```python
from build123d import *

# Parameters (mm, degrees)
CLAMP_RING_SKETCH_R          = 12.5
CLAMP_RING_25_DEPTH          = 13
CLAMP_BLOCK_DEPTH            = 13
BORE_SKETCH_R                = 6
BORE_12_DEPTH                = 13
COUNTERBORE_SKETCH_R         = 8
COUNTERBORE_16X2_DEPTH       = 2
MOUNTING_FLANGE_SKETCH_R     = 2.75
MOUNTING_FLANGE_2X_5_5_DEPTH = 7
CLAMP_SPLIT_SLOT_DEPTH       = 36.622441552
CLAMP_SCREW_HOLE_SKETCH_R    = 2.25
CLAMP_SCREW_HOLE_4_5_DEPTH   = 20


with BuildPart() as part:
    # Clamp Ring Sketch → Clamp Ring Ø25 (new body)
    with BuildSketch(Plane.XY):
        with Locations(Location((0, 0, 0), (0, 0, 180))):
            Circle(CLAMP_RING_SKETCH_R)
    extrude(amount=CLAMP_RING_25_DEPTH)

    # Clamp Block Sketch → Clamp Block (add)
    with BuildSketch(Plane.XY):
        with BuildLine():
            Line((-8.925, 22.5), (8.925, 22.5))
            Line((8.925, 22.5), (8.925, 8.751821239))
            ThreePointArc((8.925, 8.751821239), (0, 12.5), (-8.925, 8.751821239))
            Line((-8.925, 8.751821239), (-8.925, 22.5))
        make_face()
    extrude(amount=CLAMP_BLOCK_DEPTH)

    # Bore Sketch → Bore Ø12 (cut)
    with BuildSketch(Plane.XY.offset(13)):
        Circle(BORE_SKETCH_R)
    extrude(amount=-BORE_12_DEPTH, mode=Mode.SUBTRACT)

    # Counterbore Sketch → Counterbore Ø16x2 (cut)
    with BuildSketch(Plane.XY.offset(13)):
        Circle(COUNTERBORE_SKETCH_R)
    extrude(amount=-COUNTERBORE_16X2_DEPTH, mode=Mode.SUBTRACT)

    # Mounting Flange Sketch → Mounting Flange 2xØ5.5 (add)
    # profile 1 of 2: a face of its own
    with BuildSketch(Plane.XY):
        with BuildLine():
            Line((-8.925, 12.285952074), (-24.366131046, 3.44))
            Line((-24.366131046, 3.44), (-24.366131046, -3.437120562))
            Line((-24.366131046, -3.437120562), (-4.783542905, -11.548494156))
            ThreePointArc((-4.783542905, -11.548494156), (-12.247723806, -2.498651951), (-8.925, 8.751821239))
            Line((-8.925, 8.751821239), (-8.925, 12.285952074))
        make_face()
        with Locations((-18, 0)):
            Circle(MOUNTING_FLANGE_SKETCH_R, mode=Mode.SUBTRACT)
    # profile 2 of 2: a face of its own
    with BuildSketch(Plane.XY):
        with BuildLine():
            ThreePointArc((8.925, 8.751821239), (12.247723806, -2.498651951), (4.783542905, -11.548494156))
            Line((4.783542905, -11.548494156), (24.359179467, -3.44))
            Line((24.359179467, -3.44), (24.359179467, 3.44))
            Line((24.359179467, 3.44), (8.925, 12.285952074))
            Line((8.925, 12.285952074), (8.925, 8.751821239))
        make_face()
        with Locations((18, 0)):
            Circle(MOUNTING_FLANGE_SKETCH_R, mode=Mode.SUBTRACT)
    extrude(amount=MOUNTING_FLANGE_2X_5_5_DEPTH)

    # Split Slot Sketch → Clamp Split Slot (cut, through all)
    with BuildSketch(Plane.XY.offset(13)):
        with BuildLine():
            Line((0.5, 5.979130372), (0.5, 22.5))
            Line((0.5, 22.5), (-0.5, 22.5))
            Line((-0.5, 22.5), (-0.5, 5.979130372))
            ThreePointArc((-0.5, 5.979130372), (0, 6), (0.5, 5.979130372))
        make_face()
    extrude(amount=-CLAMP_SPLIT_SLOT_DEPTH, mode=Mode.SUBTRACT)

    # Clamp Screw Hole Sketch → Clamp Screw Hole Ø4.5 (cut)
    with BuildSketch(Plane(origin=(8.925, 0, 0), x_dir=(0, 0, -1), z_dir=(1, 0, 0))):
        with Locations((-6.5, 15.62591062)):
            Circle(CLAMP_SCREW_HOLE_SKETCH_R)
    extrude(amount=-CLAMP_SCREW_HOLE_4_5_DEPTH, mode=Mode.SUBTRACT)


solid = part.part
```
Can you work these out from the model? Positions are in its coordinate system, mm. A direction names the side the tool comes from. Round coordinates to 2 decimals unless told otherwise and drop trailing zeros. Loops run counter-clockwise (first coordinate to the right, second up) from the corner with the lowest first, then second, coordinate; pieces in that order, holes last. Notation, with made-up numbers: (-2, 26.25) -> (40, 26.25) arc R16 ccw to (40, 50.25) -> close; hole circle Ø9 at (18, -34.5). An arc over 180 degrees is marked (long way). Answer in a Markdown table with one row per item.
Item 1: Suppose I cut it at D-D, the plane x = 3.5. List the corners of the cut face in (y, z) for me, plus the area to 3 significant figures.
Answer block:
| item | result |
|---|---|
| outline | (-12, 0) -> (-4.87, 0) -> (-4.87, 11) -> (-7.19, 11) -> (-7.19, 13) -> (-12, 13) -> close; (4.87, 0) -> (22.5, 0) -> (22.5, 13) -> (7.19, 13) -> (7.19, 11) -> (4.87, 11) -> close; hole circle Ø4.5 at (15.63, 6.5) |
| area | 297 mm² |
Item 2: On a 3-axis mill with a long thin cutter (end or side, diameter ignored), from which of +Z, -Z, +X, -X, +Y, -Y can I reach the whole of each face in a straight line? I mean faces 5 (the flat face through (-2, -6, 11)), 6 (the flat face through (-14.712, -7.436, 3.451)). Say none if no direction works.
Answer block:
| item | result |
|---|---|
| face 5 | +Z |
| face 6 | +Z, -Z, -X, -Y |
Item 3: Suppose I cut it at B-B, the plane x = 18. List the corners of the cut face in (y, z) for me, plus the area to 3 significant figures.
Answer block:
| item | result |
|---|---|
| outline | (-6.07, 0) -> (-2.75, 0) -> (-2.75, 7) -> (-6.07, 7) -> close; (2.75, 0) -> (7.08, 0) -> (7.08, 7) -> (2.75, 7) -> close |
| area | 53.6 mm² |
Item 4: Will these pins go through, and if not, where does the flat tip stop? P1, Ø3, axis at y = 5.5, z = 10, coming from the -X side; P2, Ø3, axis at x = -6, z = 4, coming from the -Y side; P3, Ø19, axis at x = 0, y = 0, coming from the -Z side; P4, Ø1.5, axis at y = 18, z = 2, coming from the +X side (3 decimals).
Answer block:
| item | result |
|---|---|
| P1 | x = -11.84 |
| P2 | y = -11.66 |
| P3 | z = 0 |
| P4 | x = 8.925 |
Item 5: If I drill on probe 1 along X at (y, z) = (13, 4.5) (3 decimals); probe 2 along X at (y, z) = (0, 11.8); probe 3 along Y at (x, z) = (3, 6.5), over which ranges is the centre line in solid material (lowest first)?
Answer block:
| item | result |
|---|---|
| probe 1 | -8.925 to -0.5, 0.5 to 8.925 |
| probe 2 | -12.5 to -8, 8 to 12.5 |
| probe 3 | -12.13 to -5.2, 5.2 to 13.38, 17.88 to 22.5 |
Item 6: Suppose I cut it at C-C, the plane y = 0.5. List the corners of the cut face in (x, z) for me.
Answer block:
| item | result |
|---|---|
| outline | (-24.37, 0) -> (-20.7, 0) -> (-20.7, 7) -> (-24.37, 7) -> close; (-15.3, 0) -> (-5.98, 0) -> (-5.98, 11) -> (-7.98, 11) -> (-7.98, 13) -> (-12.49, 13) -> (-12.49, 7) -> (-15.3, 7) -> close; (5.98, 0) -> (15.3, 0) -> (15.3, 7) -> (12.49, 7) -> (12.49, 13) -> (7.98, 13) -> (7.98, 11) -> (5.98, 11) -> close; (20.7, 0) -> (24.36, 0) -> (24.36, 7) -> (20.7, 7) -> close |
Item 7: Suppose I cut it at A-A, the plane z = 6.5. Give the number of separate pieces and of enclosed holes in the cut face, plus the area to 3 significant figures.
Answer block:
| item | result |
|---|---|
| separate pieces | 3 |
| enclosed holes | 2 |
| area | 801 mm² |
Item 8: We'd pull the mould along X, two halves only. Please class faces 1 (the cylindrical face through (-0.411, -12.493, 9.298)), 2 (the flat face through (-8.925, 19, 6)), 3 (the flat face through (-0.5, 13, 7)), 4 (the flat face through (14.434, -7.551, 3.451)): released by +X, released by -X, zero draft, split by the parting line, or undercut.
Answer block:
| item | result |
|---|---|
| face 1 | split by the parting line |
| face 2 | released by -X |
| face 3 | undercut |
| face 4 | released by +X |
